```python
from build123d import *

# Parameters (mm, degrees)
SKETCH_1_R      = 24
EXTRUDE_1_DEPTH = 15
M10X1_0_1_D     = 9
M10X1_0_1_DEPTH = 20
M10X1_0_1_TIP   = 2.703872786
CHAMFER_1_SIZE  = 1


with BuildPart() as part:
    # 草图1 → 凸台-拉伸1 (new, symmetric)
    with BuildSketch(Plane(origin=(0, 0, 0), x_dir=(0, 0, -1), z_dir=(1, 0, 0))):
        with BuildLine():
            Line((-750, -35), (750, -35))
            ThreePointArc((750, -35), (785, 0), (750, 35))
            Line((750, 35), (-750, 35))
            ThreePointArc((-750, 35), (-785, 0), (-750, -35))
        make_face()
        with Locations((-750, 0)):
            Circle(SKETCH_1_R, mode=Mode.SUBTRACT)
        with Locations((750, 0)):
            Circle(SKETCH_1_R, mode=Mode.SUBTRACT)
    extrude(amount=EXTRUDE_1_DEPTH, both=True)

    # M10x1.0 螺纹孔1
    with Locations(Plane(origin=(0, 35, 0), x_dir=(1, 0, 0), z_dir=(0, 1, 0))):
        with Locations((0, -750), (0, 750)):
            Hole(M10X1_0_1_D / 2, depth=M10X1_0_1_DEPTH)
            with Locations((0, 0, -(M10X1_0_1_DEPTH + M10X1_0_1_TIP / 2))):  # 118° drill point
                Cone(0, M10X1_0_1_D / 2, M10X1_0_1_TIP, mode=Mode.SUBTRACT)

    # 倒角1
    chamfer_1_edges = [part.edges().sort_by_distance(p)[0] for p in [
        (-15, 0, 774),
        (15, 0, 774),
        (-15, 0, -726),
        (15, 0, -726),
    ]]
    chamfer(chamfer_1_edges, length=CHAMFER_1_SIZE)


solid = part.part
```
Part model, mm, in its own coordinate system. Round coordinates to 2 decimals unless told otherwise and drop trailing zeros. Loops run counter-clockwise (first coordinate to the right, second up) from the corner with the lowest first, then second, coordinate; pieces in that order, holes last.
Item 1: Cut at A-A, the plane y = 0. Give the cut face in (x, z), then the cut area to 3 significant figures.
Item 2: Mould opens along Y. For faces 1 (the face through (15, 0, 11)), 2 (the face through (0.21, 0.77, 784.99)), 3 (the face through (-0.2, -23.43, -744.8)) say: +Y half, -Y half, draft (parallel to the pull), parting line (faces both ways), or undercut.
Item 3: Drill centre lines: line 1 (Z direction, x = -2.5, y = -3.5); line 2 (Z direction, x = 6, y = -6.5); line 3 (X direction, y = 28, z = -750). Where is each one in solid material? Low to high.
Item 4: Drop flat-ended pins along their axis: P1, Ø8, axis at x = -4.5, y = 0, coming from the -Z side; P2, Ø1.5, axis at x = 1, y = 22, coming from the -Z side; P3, Ø6, axis at x = -9, y = 10.5, coming from the -Z side. Give the stop position or say it passes through.
A:
1. outline: (-15, -785) - (15, -785) - (15, -775) - (14, -774) - (-14, -774) - (-15, -775) - close; (-15, -725) - (-14, -726) - (14, -726) - (15, -725) - (15, 725) - (14, 726) - (-14, 726) - (-15, 725) - close; (-15, 775) - (-14, 774) - (14, 774) - (15, 775) - (15, 785) - (-15, 785) - close
1. area: 44,200 mm2
2. face 1: draft
2. face 2: parting line
2. face 3: undercut
3. line 1: z = -784.82 to -773.74, -726.26 to 726.26, 773.74 to 784.82
3. line 2: z = -784.39 to -773.1, -726.9 to 726.9, 773.1 to 784.39
3. line 3: x = -15 to -4.5, 4.5 to 15
4. P1: stops at z = -785
4. P2: stops at z = -777.81
4. P3: stops at z = -784.19
